```python
from build123d import *

# Parameters (mm, degrees)
SKETCH1_W              = 330
SKETCH1_H              = 100
BOSS_EXTRUDE1_DEPTH    = 10
M12_TAPPED_HOLE1_D     = 10.2
M12_TAPPED_HOLE1_DEPTH = 29.25
M12_TAPPED_HOLE1_TIP   = 3.064389157


with BuildPart() as part:
    # Sketch1 → Boss-Extrude1 (new body)
    with BuildSketch(Plane.XY):
        Rectangle(SKETCH1_W, SKETCH1_H)
    extrude(amount=BOSS_EXTRUDE1_DEPTH)

    # M12 Tapped Hole1
    with Locations(Plane.XY.offset(10)):
        with Locations((-125, 0), (-80, 8), (-80, 28), (80, 28), (80, 8), (125, 0)):
            Hole(M12_TAPPED_HOLE1_D / 2, depth=M12_TAPPED_HOLE1_DEPTH)
            with Locations((0, 0, -(M12_TAPPED_HOLE1_DEPTH + M12_TAPPED_HOLE1_TIP / 2))):  # 118° drill point
                Cone(0, M12_TAPPED_HOLE1_D / 2, M12_TAPPED_HOLE1_TIP, mode=Mode.SUBTRACT)


solid = part.part
```
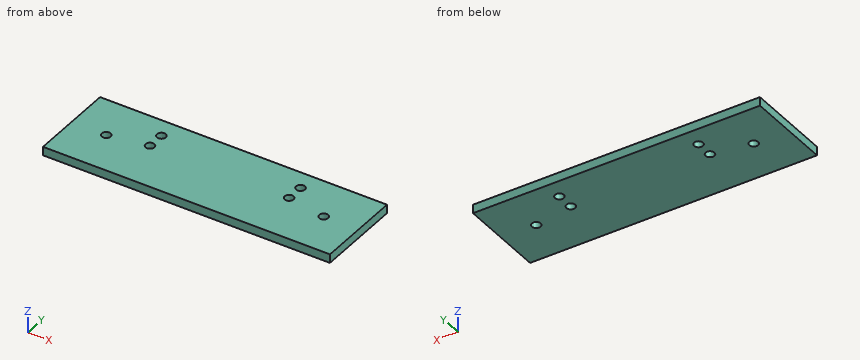
Geometry check sheet. Reference: the model listing, model coordinates, mm. Give positions to 0.01 mm unless a question says otherwise; leave off trailing zeros. Loops run counter-clockwise (first coordinate to the right, second up) from the corner with the lowest first, then second, coordinate; pieces in that order, holes last. Notation, with made-up numbers: M 77,84.25 L 88,84.25 A24 cw 88,122.25 Z; hole C 75,31.5 d6. An arc over 180 degrees is marked long. Answer as CSV lines item,"result".
Item 1: Cross-section at A-A on y = 8. Record the cut outline in (x, z).
Values:
outline,"M -165,0 L -85.1,0 L -85.1,10 L -165,10 Z; M -74.9,0 L 74.9,0 L 74.9,10 L -74.9,10 Z; M 85.1,0 L 165,0 L 165,10 L 85.1,10 Z"
Item 2: Cross-section at B-B on x = 125. Record the cut outline in (y, z).
Values:
outline,"M -50,0 L -5.1,0 L -5.1,10 L -50,10 Z; M 5.1,0 L 50,0 L 50,10 L 5.1,10 Z"
Item 3: Cross-section at C-C on x = -80. Record the cut outline in (y, z), and give its area (3 significant figures).
Values:
outline,"M -50,0 L 2.9,0 L 2.9,10 L -50,10 Z; M 13.1,0 L 22.9,0 L 22.9,10 L 13.1,10 Z; M 33.1,0 L 50,0 L 50,10 L 33.1,10 Z"
area,"796 mm²"
Item 4: Depth check by flat-ended pin: P1, Ø11.5, axis at x = -80, y = 28, coming from the +Z side; P2, Ø6, axis at x = 125, y = 0, coming from the +Z side. Enter the tip coordinate at first touch or a pass-through.
Values:
P1,"stops at z = 10"
P2,"passes through"
Item 5: Material ranges on line 1 (Y direction, x = 80, z = 3.25); line 2 (X direction, y = 1, z = 5); line 3 (Y direction, x = -125, z = 7), recorded low to high.
Values:
line 1,"y = -50 to 2.9, 13.1 to 22.9, 33.1 to 50"
line 2,"x = -165 to -130, -120 to 120, 130 to 165"
line 3,"y = -50 to -5.1, 5.1 to 50"
